The model under review builds one solid part; all positions refer to its coordinate system, in mm. Face numbers are marked on the shaded views. A direction names the side the tool comes from. Give positions to 0.01 mm unless a question says otherwise; leave off trailing zeros. Order: outer loops, then holes, each group sorted by start corner. A loop starts at its lowest first (then second) coordinate and runs counter-clockwise, first axis right, second up. Notation, with made-up numbers: (-9, 30) - (23, 30) arc R19 ccw to (23, 39) - close; hole circle Ø4 at (66.5, -40). An arc over 180 degrees is marked (long way). Use CSV: the item, a comma, the result in double quotes.
```python
from build123d import *

# Parameters (mm, degrees)
SKETCH1_R             = 24
BOSS_EXTRUDE1_DEPTH   = 12
SKETCH2_R             = 20
BOSS_EXTRUDE2_DEPTH   = 2
SKETCH3_R             = 17.5
BOSS_EXTRUDE3_DEPTH   = 27
SKETCH4_R             = 13
BOSS_EXTRUDE4_DEPTH   = 15
SKETCH5_R             = 14
CUT_EXTRUDE1_DEPTH    = 37.1
SKETCH6_R             = 8.25
CUT_EXTRUDE2_DEPTH    = 66.482822175
CUT_EXTRUDE3_DEPTH    = 4
CUT_EXTRUDE4_START    = -7.5
SKETCH8_R             = 29.21642444
SKETCH8_R_2           = 16.5
CUT_EXTRUDE4_DEPTH    = 1.5
M5_TAPPED_HOLE1_D     = 4.2
M5_TAPPED_HOLE1_DEPTH = 10
M5_TAPPED_HOLE1_TIP   = 1.2618073
CHAMFER1_SIZE         = 0.5


with BuildPart() as part:
    # Sketch1 → Boss-Extrude1 (new body)
    with BuildSketch(Plane.XY):
        Circle(SKETCH1_R)
    extrude(amount=BOSS_EXTRUDE1_DEPTH)

    # Sketch2 → Boss-Extrude2 (add)
    with BuildSketch(Plane.XY.offset(12)):
        Circle(SKETCH2_R)
    extrude(amount=BOSS_EXTRUDE2_DEPTH)

    # Sketch3 → Boss-Extrude3 (add)
    with BuildSketch(Plane.XY.offset(14)):
        Circle(SKETCH3_R)
    extrude(amount=BOSS_EXTRUDE3_DEPTH)

    # Sketch4 → Boss-Extrude4 (add)
    with BuildSketch(Plane.XY.offset(41)):
        Circle(SKETCH4_R)
    extrude(amount=BOSS_EXTRUDE4_DEPTH)

    # Sketch5 → Cut-Extrude1 (cut)
    with BuildSketch(Plane(origin=(0, 0, 0), x_dir=(-1, 0, 0), z_dir=(0, 0, -1))):
        Circle(SKETCH5_R)
    extrude(amount=-CUT_EXTRUDE1_DEPTH, mode=Mode.SUBTRACT)

    # Sketch6 → Cut-Extrude2 (cut, through all)
    with BuildSketch(Plane.XY.offset(56)):
        Circle(SKETCH6_R)
    extrude(amount=-CUT_EXTRUDE2_DEPTH, mode=Mode.SUBTRACT)

    # Sketch7 → Cut-Extrude3 (cut)
    with BuildSketch(Plane(origin=(0, 13, 0), x_dir=(1, 0, 0), z_dir=(0, 1, 0))):
        with BuildLine():
            Line((4, -48), (4, -64))
            ThreePointArc((4, -64), (0, -68), (-4, -64))
            Line((-4, -64), (-4, -48))
            ThreePointArc((-4, -48), (0, -44), (4, -48))
        make_face()
    extrude(amount=-CUT_EXTRUDE3_DEPTH, mode=Mode.SUBTRACT)

    # Sketch8 → Cut-Extrude4 (cut)
    with BuildSketch(Plane.XY.offset(41).offset(CUT_EXTRUDE4_START)):
        Circle(SKETCH8_R)
        Circle(SKETCH8_R_2, mode=Mode.SUBTRACT)
    extrude(amount=-CUT_EXTRUDE4_DEPTH, mode=Mode.SUBTRACT)

    # M5 Tapped Hole1
    with Locations(Plane(origin=(0, 0, 0), x_dir=(-1, 0, 0), z_dir=(0, 0, -1))):
        with Locations((0, 19), (-13.435028843, 13.435028843), (13.435028843, 13.435028843), (-13.435028843, -13.435028843), (0, -19), (13.435028843, -13.435028843)):
            Hole(M5_TAPPED_HOLE1_D / 2, depth=M5_TAPPED_HOLE1_DEPTH)
            with Locations((0, 0, -(M5_TAPPED_HOLE1_DEPTH + M5_TAPPED_HOLE1_TIP / 2))):  # 118° drill point
                Cone(0, M5_TAPPED_HOLE1_D / 2, M5_TAPPED_HOLE1_TIP, mode=Mode.SUBTRACT)

    # Chamfer1
    chamfer1_edges = [part.edges().sort_by_distance(p)[0] for p in [
        (-17.5, 0, 41),
        (-24, 0, 0),
        (-7.64852927, -10.511898021, 56),
        (-24, 0, 12),
    ]]
    chamfer(chamfer1_edges, length=CHAMFER1_SIZE)


solid = part.part
```
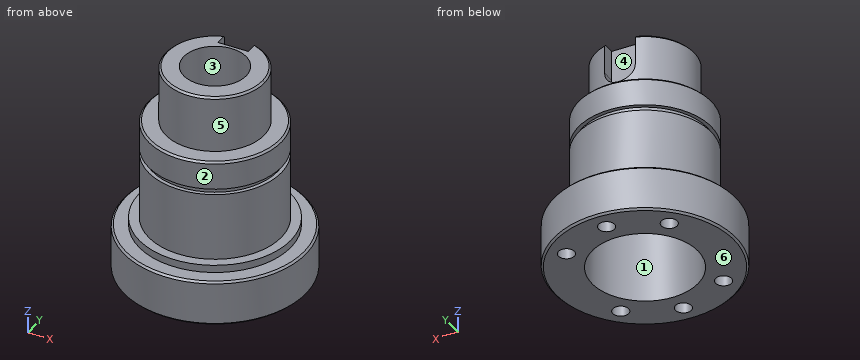
Item 1: Mouldability with a two-part tool opening along Y and no side actions: class the marked faces 1, 2, 3 and 4 as pulls with the +Y half, pulls with the -Y half, needs draft (parallel to the pull), parting line crosses it, or undercut.
Results list:
face 1,"undercut"
face 2,"parting line crosses it"
face 3,"undercut"
face 4,"pulls with the +Y half"
Item 2: Take a section at A-A, the plane z = 17.5. Give the boundary of the cut face in (x, y).
Results list:
outline,"circle Ø35 at (0, 0); hole circle Ø28 at (0, 0)"
Item 3: Clearance check with flat-ended pins moving along their axes: pin 1 (4 mm diameter, centred on y = -7.5, z = 29, fed in from -X); pin 2 (4 mm diameter, centred on x = 0.5, z = 50.5, fed in from +Y); pin 3 (1 mm diameter, centred on y = -14, z = 46, fed in from +X); pin 4 (2.5 mm diameter, centred on y = 11, z = 50, fed in from +X). State where each tip first meets the part, or that it passes through.
Results list:
pin 1,"stops at x = -16.61"
pin 2,"stops at y = 9"
pin 3,"passes through"
pin 4,"stops at x = 8.6"
Item 4: Wall thickness on L1, parallel to Y at x = 0, z = 47.25; L2, parallel to Y at x = 0, z = 43; L3, parallel to Z at x = -14, y = -9: over which ranges is each line inside the solid? List them lowest first.
Results list:
L1,"y = -13 to -8.25, 8.25 to 9"
L2,"y = -13 to -8.25, 8.25 to 13"
L3,"z = 0 to 32, 33.5 to 41"
Item 5: Tool access review of the marked faces 5 and 6: name each direction out of +Z, -Z, +X, -X, +Y, -Y from which nothing blocks a thin tool from reaching the whole face with its end or side.
Results list:
face 5,"+Z"
face 6,"-Z, +X, -X, +Y, -Y"
